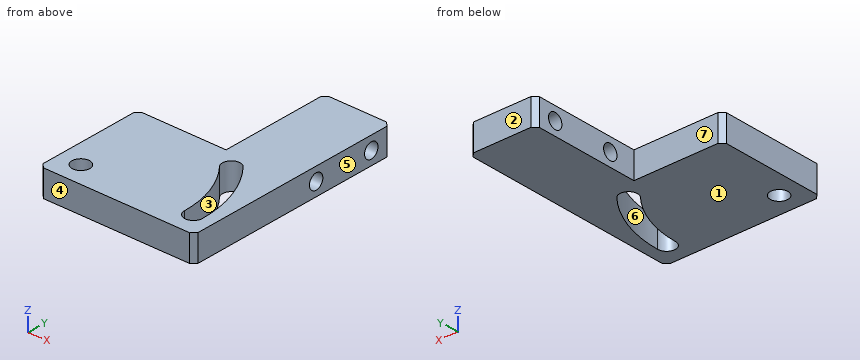
from build123d import *

# Parameters (mm, degrees)
SKETCH_1_W          = 35
SKETCH_1_H          = 50
EXTRUDE_1_DEPTH     = 3
SKETCH_2_W          = 20
SKETCH_2_H          = 25
CUT_EXTRUDE_1_DEPTH = 32.10064308
SKETCH_3_R          = 2
CUT_EXTRUDE_2_DEPTH = 32.10064308
HOLE_WIZARD_M3_1_D  = 3.4
CHAMFER_1_SIZE      = 1


with BuildPart() as part:
    # 草图1 → 凸台-拉伸1 (new, symmetric)
    with BuildSketch(Plane.XY):
        Rectangle(SKETCH_1_W, SKETCH_1_H)
    extrude(amount=EXTRUDE_1_DEPTH, both=True)

    # 草图2 → 切除-拉伸1 (cut, through all)
    with BuildSketch(Plane.XY.offset(3)):
        with Locations((-7.5, 12.5)):
            Rectangle(SKETCH_2_W, SKETCH_2_H)
    extrude(amount=-CUT_EXTRUDE_1_DEPTH, mode=Mode.SUBTRACT)

    # 草图3 → 切除-拉伸2 (cut, through all)
    with BuildSketch(Plane.XY.offset(3)):
        with Locations((-12.5, -20)):
            Circle(SKETCH_3_R)
        with BuildLine():
            ThreePointArc((14.9, -20), (13.24757781, -10.628648073), (8.489617741, -2.387619495))
            ThreePointArc((8.489617741, -2.387619495), (5.671953636, -2.141105828), (5.425439969, -4.958769933))
            ThreePointArc((5.425439969, -4.958769933), (9.488807326, -11.996728646), (10.9, -20))
            ThreePointArc((10.9, -20), (12.9, -22), (14.9, -20))
        make_face()
    extrude(amount=-CUT_EXTRUDE_2_DEPTH, mode=Mode.SUBTRACT)

    # M3 间隙孔1 (through all)
    with Locations(Plane.ZY.offset(-2.5)):
        with Locations((0, 20), (0, 6)):
            Hole(HOLE_WIZARD_M3_1_D / 2)

    # 倒角1
    chamfer_1_edges = [part.edges().sort_by_distance(p)[0] for p in [
        (-17.5, 0, 0),
        (2.5, 25, 0),
        (17.5, 25, 0),
        (17.5, -25, 0),
        (-17.5, -25, 0),
    ]]
    chamfer(chamfer_1_edges, length=CHAMFER_1_SIZE)


solid = part.part
Work out the finished part from the listing and answer in its coordinate system (mm). Face numbers are marked on the shaded views. A direction names the side the tool comes from. Coordinates: 2 decimals unless noted, no trailing zeros. Loops run counter-clockwise (first coordinate to the right, second up) from the corner with the lowest first, then second, coordinate; pieces in that order, holes last. Notation, with made-up numbers: (7, 47.25) -> (54, 47.25) arc R36 cw to (54, 81.25) -> close; hole circle Ø9 at (9.25, -4.5). An arc over 180 degrees is marked (long way). Answer as CSV lines item,"result".
1) The part is cut by section A-A (x = 13.5). Give the vertices of the cut face in (y, z), and give its area (3 significant figures).
A:
outline,"(-25, -3) -> (-21.91, -3) -> (-21.91, 3) -> (-25, 3) -> close; (-11.35, -3) -> (25, -3) -> (25, 3) -> (-11.35, 3) -> close; hole circle Ø3.4 at (6, 0); hole circle Ø3.4 at (20, 0)"
area,"219 mm²"
2) For a pull along Y with two mould halves and no side action, classify the marked faces 1, 2, 3 and 4 as released by +Y, released by -Y, zero draft, split by the parting line, or undercut.
A:
face 1,"zero draft"
face 2,"released by +Y"
face 3,"undercut"
face 4,"released by -Y"
3) The part is cut by section C-C (z = -0.5). Give the vertices of the cut face in (x, y).
A:
outline,"(-17.5, -24) -> (-16.5, -25) -> (16.5, -25) -> (17.5, -24) -> (17.5, 4.38) -> (2.5, 4.38) -> (2.5, 0) -> (-16.5, 0) -> (-17.5, -1) -> close; (2.5, 7.62) -> (17.5, 7.62) -> (17.5, 18.38) -> (2.5, 18.38) -> close; (2.5, 21.62) -> (17.5, 21.62) -> (17.5, 24) -> (16.5, 25) -> (3.5, 25) -> (2.5, 24) -> close; hole circle Ø4 at (-12.5, -20); hole (5.43, -4.96) arc R23.4 cw to (10.9, -20) arc R2 ccw to (14.9, -20) arc R27.4 ccw to (8.49, -2.39) arc R2 ccw to start"
4) For the marked faces 5, 6 and 7, determine the directions among +Z, -Z, +X, -X, +Y, -Y from which every point of the face is accessible in a straight line to the end or side of a thin tool.
A:
face 5,"+Z, -Z, +X, +Y, -Y"
face 6,"+Z, -Z"
face 7,"+Z, -Z, -X, +Y"
5) The part is cut by section B-B (y = 6). Give the vertices of the cut face in (x, z), and give its area (3 significant figures).
A:
outline,"(2.5, -3) -> (17.5, -3) -> (17.5, -1.7) -> (2.5, -1.7) -> close; (2.5, 1.7) -> (17.5, 1.7) -> (17.5, 3) -> (2.5, 3) -> close"
area,"39.0 mm²"
6) Straight lines are drawn through the part: probe 1 along X at (y, z) = (-21.5, 0.6); probe 2 along Y at (x, z) = (-12.5, -1.2); probe 3 along X at (y, z) = (6.5, -1.7). For each, find the intervals that lie inside material, in ascending order.
A:
probe 1,"x = -17.5 to -13.82, -11.18 to 11.58, 14.22 to 17.5"
probe 2,"y = -25 to -22, -18 to 0"
probe 3,"x = 2.5 to 17.5"
7) Flat-ended cylindrical pins translate along their axes: pin 1 (3 mm diameter, centred on y = 14, z = -1, fed in from -X); pin 2 (2.5 mm diameter, centred on y = 20, z = 0, fed in from -X). Find the tip coordinate at first contact, or state that the pin passes through.
A:
pin 1,"stops at x = 2.5"
pin 2,"passes through"
8) The part is cut by section D-D (x = 3). Give the vertices of the cut face in (y, z).
A:
outline,"(-25, -3) -> (24.5, -3) -> (24.5, 3) -> (-25, 3) -> close; hole circle Ø3.4 at (6, 0); hole circle Ø3.4 at (20, 0)"
